```python
from build123d import *

# Parameters (mm, degrees)
SKETCH2_R           = 10
BOSS_EXTRUDE1_DEPTH = 8
CUT_EXTRUDE1_DEPTH  = 10


with BuildPart() as part:
    # Sketch2 → Boss-Extrude1 (new body)
    with BuildSketch(Plane.XY):
        with BuildLine():
            Line((-16.639082443, 618.903111451), (-80, 713.908799417))
            Line((-80, 713.908799417), (-80, 1100.091200583))
            Line((-80, 1100.091200583), (-16.639082443, 1195.096888549))
            ThreePointArc((-16.639082443, 1195.096888549), (0, 1204), (16.639082443, 1195.096888549))
            Line((16.639082443, 1195.096888549), (80, 1100.091200583))
            Line((80, 1100.091200583), (80, 713.908799417))
            Line((80, 713.908799417), (16.639082443, 618.903111451))
            ThreePointArc((16.639082443, 618.903111451), (0, 610), (-16.639082443, 618.903111451))
        make_face()
        with Locations((0, 630)):
            Circle(SKETCH2_R, mode=Mode.SUBTRACT)
    extrude(amount=BOSS_EXTRUDE1_DEPTH)

    # Sketch4 → Cut-Extrude1 (cut)
    with BuildSketch(Plane.XY.offset(8)):
        with BuildLine():
            Line((-49.84926833, 770.742207295), (-47.561478164, 770.742207295))
            ThreePointArc((-47.561478164, 770.742207295), (0, 793.027742088), (47.561478164, 770.742207295))
            Line((47.561478164, 770.742207295), (49.84926833, 770.742207295))
            ThreePointArc((49.84926833, 770.742207295), (54.413886924, 773.70155615), (53.575185994, 779.076504457))
            ThreePointArc((53.575185994, 779.076504457), (0, 803.027742088), (-53.575185994, 779.076504457))
            ThreePointArc((-53.575185994, 779.076504457), (-54.413886924, 773.70155615), (-49.84926833, 770.742207295))
        make_face()
    extrude(amount=-CUT_EXTRUDE1_DEPTH, mode=Mode.SUBTRACT)


solid = part.part
```
Check sheet for the modelled part. Datum: model origin and axes. Units: mm. A direction names the side the tool comes from. Give positions to 0.01 mm unless a question says otherwise; leave off trailing zeros. Write each loop counter-clockwise with the first axis right and the second up, starting at its lowest first coordinate (ties: lowest second). Pieces come first, ordered by that corner, then holes.
Item 1: Cross-section at A-A (x = 0). Enter the section's corners in (y, z), and give its area (3 significant figures).
Item 2: Cross-section at D-D (y = 630). Enter the section's corners in (x, z), and give its area (3 significant figures).
Item 3: Draft check along X on faces 1 (the face through (0.846, 803.023, 4.056)), 2 (the face through (-1.302, 639.915, 3.944)), 3 (the face through (48.76, 667.07, 3.94)), 4 (the face through (1, 911, 8)). Enter one of: released by +X, released by -X, zero draft, split by the parting line, or undercut.
Item 4: Scan lines: L1, parallel to Y at x = 0, z = 4.25; L2, parallel to Y at x = 5.5, z = 6.25; L3, parallel to X at y = 630, z = 3.5. Record each from-to range of solid material in increasing order.
Item 5: Cross-section at B-B (z = 1.5). Enter the section's corners in (x, y), and give its area (3 significant figures).
Item 6: Cross-section at C-C (x = 31.5). Enter the section's corners in (y, z).
Item 7: Access from +Z, -Z, +X, -X, +Y, -Y to the whole of each face (thin tool, end or side, straight path). Record for faces 5 (the face through (-0.759, 793.023, 4.056)), 6 (the face through (1, 911, 0)).
Item 8: Gauge pin test, flat ends, axial feed: pin 1 (3 mm diameter, centred on x = 15, z = 5.5, fed in from -Y); pin 2 (2.5 mm diameter, centred on x = -48.5, z = 2.5, fed in from +Y); pin 3 (2 mm diameter, centred on x = -19, y = 791.5, fed in from -Z); pin 4 (2.5 mm diameter, centred on x = 49, z = 3, fed in from +Y). Record the tip position at first contact, or that the pin passes through.
Report:
1. outline: (610, 0) - (620, 0) - (620, 8) - (610, 8) - close; (640, 0) - (793.03, 0) - (793.03, 8) - (640, 8) - close; (803.03, 0) - (1204, 0) - (1204, 8) - (803.03, 8) - close
1. area: 4,510 mm2
2. outline: (-24.04, 0) - (-10, 0) - (-10, 8) - (-24.04, 8) - close; (10, 0) - (24.04, 0) - (24.04, 8) - (10, 8) - close
2. area: 225 mm2
3. face 1: undercut
3. face 2: undercut
3. face 3: released by +X
3. face 4: zero draft
4. L1: y = 610 to 620, 640 to 793.03, 803.03 to 1204
4. L2: y = 610.77 to 621.65, 638.35 to 792.78, 802.82 to 1203.23
4. L3: x = -24.04 to -10, 10 to 24.04
5. outline: (-80, 713.91) - (-16.64, 618.9) arc R20 ccw to (16.64, 618.9) - (80, 713.91) - (80, 1100.09) - (16.64, 1195.1) arc R20 ccw to (-16.64, 1195.1) - (-80, 1100.09) - close; hole (-53.58, 779.08) arc R5 ccw to (-49.85, 770.74) - (-47.56, 770.74) arc R61.9 cw to (47.56, 770.74) - (49.85, 770.74) arc R5 ccw to (53.58, 779.08) arc R71.9 ccw to start; hole circle Ø20 at (0, 630)
5. area: 79,000 mm2
6. outline: (641.19, 0) - (784.41, 0) - (784.41, 8) - (641.19, 8) - close; (795.76, 0) - (1172.81, 0) - (1172.81, 8) - (795.76, 8) - close
7. face 5: +Z, -Z
7. face 6: -Z, +X, -X, +Y, -Y
8. pin 1: stops at y = 615.24
8. pin 2: stops at y = 1149.2
8. pin 3: passes through
8. pin 4: stops at y = 1148.45
